Verification items for the finished model (mm, model axes). Give positions to 0.01 mm unless a question says otherwise; leave off trailing zeros. Loops run counter-clockwise (first coordinate to the right, second up) from the corner with the lowest first, then second, coordinate; pieces in that order, holes last. Notation, with made-up numbers: (1, -24) - (56, -24) arc R19 cw to (56, 3) - close; hole circle Ø7 at (28, 3). An arc over 180 degrees is marked (long way). Use one line per item in the form item = value.
```python
from build123d import *
from OCP.BRepFilletAPI import BRepFilletAPI_MakeChamfer

# Parameters (mm, degrees)
SKETCH1_R                                            = 14
BOSS_EXTRUDE1_DEPTH                                  = 3.5
CHAMFER1_SIZE                                        = 0.5
CHAMFER1_SIZE2                                       = 0.288675135
CSK_FOR_M6_HEXAGON_LOBULAR_SOCKET_RAISED_D           = 6.6
CSK_FOR_M6_HEXAGON_LOBULAR_SOCKET_RAISED_DEPTH       = 6.5
CSK_FOR_M6_HEXAGON_LOBULAR_SOCKET_RAISED_CSINK_D     = 12.8
CSK_FOR_M6_HEXAGON_LOBULAR_SOCKET_RAISED_CSINK_ANGLE = 90
CSK_FOR_M6_HEXAGON_LOBULAR_SOCKET_RAISED_TIP         = 1.982840043


with BuildPart() as part:
    # Sketch1 → Boss-Extrude1 (new body)
    with BuildSketch(Plane.XY):
        Circle(SKETCH1_R)
    extrude(amount=BOSS_EXTRUDE1_DEPTH)

    # Chamfer1: one chamfer whose edges measure the first distance from different faces: ONE call of the kernel's chamfer builder (chamfer() names one face for all edges)
    chamfer1_edges_1 = [part.edges().sort_by_distance(p)[0] for p in [
        (-14, 0, 0),
    ]]
    chamfer1_side_1 = [part.faces().sort_by_distance(p)[0] for p in [
        (0, 0, 0),
    ]]
    chamfer1_edges_2 = [part.edges().sort_by_distance(p)[0] for p in [
        (-14, 0, 3.5),
    ]]
    chamfer1_side_2 = [part.faces().sort_by_distance(p)[0] for p in [
        (-14, 0, 1.75),
    ]]
    chamfer1 = BRepFilletAPI_MakeChamfer(part.part.solid().wrapped)
    for e in chamfer1_edges_1:
        chamfer1.Add(CHAMFER1_SIZE, CHAMFER1_SIZE2, e.wrapped, chamfer1_side_1[0].wrapped)  # the first distance lies on this face
    for e in chamfer1_edges_2:
        chamfer1.Add(CHAMFER1_SIZE, CHAMFER1_SIZE2, e.wrapped, chamfer1_side_2[0].wrapped)  # the first distance lies on this face
    add(Compound.cast(chamfer1.Shape()), mode=Mode.REPLACE)

    # CSK for M6 Hexagon lobular socket raised CTSK head screws1
    with Locations(Plane(origin=(0.028531749, 0.017266162, 0), x_dir=(-1, 0, 0), z_dir=(0, 0, -1))):
        with Locations((0, 0)):
            CounterSinkHole(CSK_FOR_M6_HEXAGON_LOBULAR_SOCKET_RAISED_D / 2, CSK_FOR_M6_HEXAGON_LOBULAR_SOCKET_RAISED_CSINK_D / 2, depth=CSK_FOR_M6_HEXAGON_LOBULAR_SOCKET_RAISED_DEPTH, counter_sink_angle=CSK_FOR_M6_HEXAGON_LOBULAR_SOCKET_RAISED_CSINK_ANGLE)
            with Locations((0, 0, -(CSK_FOR_M6_HEXAGON_LOBULAR_SOCKET_RAISED_DEPTH + CSK_FOR_M6_HEXAGON_LOBULAR_SOCKET_RAISED_TIP / 2))):  # 118° drill point
                Cone(0, CSK_FOR_M6_HEXAGON_LOBULAR_SOCKET_RAISED_D / 2, CSK_FOR_M6_HEXAGON_LOBULAR_SOCKET_RAISED_TIP, mode=Mode.SUBTRACT)


solid = part.part
```
1. Scan lines: probe 1 along X at (y, z) = (1, 0.3); probe 2 along X at (y, z) = (-2, 1.7); probe 3 along Y at (x, z) = (2.5, 1.9). Record each from-to range of solid material in increasing order.
Result set:
probe_1 = -13.96 to -5.99, 6.05 to 13.96
probe_2 = -13.86 to -4.22, 4.27 to 13.86
probe_3 = -13.77 to -3.74, 3.78 to 13.77
2. Depth check by flat-ended pin: pin 1 Ø2 at (x, z) = (-7.5, 1.5) entering from +Y; pin 2 Ø8.5 at (x, y) = (0.03, 0.02) entering from +Z. Enter the tip coordinate at first touch or a pass-through.
Result set:
pin_1 = 12.4
pin_2 = 3.5
3. Draft check along Y on faces 1 (the cylindrical face through (12.932, -5.362, 1.625)), 2 (the flat face through (3, -3, 3.5)), 3 (the cylindrical face through (-0.7, -3.2, 3.3)). Enter one of: released by +Y, released by -Y, zero draft, split by the parting line, or undercut.
Result set:
face_1 = split by the parting line
face_2 = zero draft
face_3 = undercut
4. Section check A-A, the plane z = 2.3. Record the cut outline in (x, y).
Result set:
outline = circle Ø28 at (0, 0); hole circle Ø8.2 at (0.03, 0.02)
